Build history of the part. All positions in model axes, mm. A direction names the side the tool comes from. Coordinates: 2 decimals unless noted, no trailing zeros. Loops run counter-clockwise (first coordinate to the right, second up) from the corner with the lowest first, then second, coordinate; pieces in that order, holes last. Notation, with made-up numbers: (59, 86) - (94, 86) arc R18 ccw to (94, 113) - close; hole circle Ø1 at (3, -28.75). An arc over 180 degrees is marked (long way). One line per item, written item: value.
```python
from build123d import *

# Parameters (mm, degrees)
BOSS_EXTRUDE2_DEPTH = 45


with BuildPart() as part:
    # Sketch1 → Boss-Extrude2 (new body)
    with BuildSketch(Plane.XY):
        Polygon((-15.25, 11.25), (-14.75, 11.75), (-8, 11.75), (-8, 10.25), (-5, 10.25), (-5, 11.75), (5, 11.75), (5, 10.25), (8, 10.25), (8, 11.75), (14.75, 11.75), (15.25, 11.25), (15.25, 2.78649269), (13.75, 2.78649269), (13.75, -2.78649269), (15.25, -2.78649269), (15.25, -11.25), (14.75, -11.75), (8, -11.75), (8, -10.25), (5, -10.25), (5, -11.75), (-5, -11.75), (-5, -10.25), (-8, -10.25), (-8, -11.75), (-14.75, -11.75), (-15.25, -11.25), (-15.25, -2.78649269), (-13.75, -2.78649269), (-13.75, 2.78649269), (-15.25, 2.78649269), align=None)
    extrude(amount=BOSS_EXTRUDE2_DEPTH)


solid = part.part
```
Item 1: Pull direction Y, two halves, no side cores. Call faces 6 (the face through (15, 2.786, 22)), 7 (the face through (-13.75, 0, 22)), 8 (the face through (-11, 11.75, 22)), 9 (the face through (-5, -11, 22)): released by +Y, released by -Y, zero draft, split by the parting line, or undercut.
Check result:
face 6: undercut
face 7: undercut
face 8: released by +Y
face 9: zero draft
Item 2: Probe probe 1 along X at (y, z) = (-0.25, 36); probe 2 along Y at (x, z) = (-7, 4.5). List the from-to ranges inside material, lowest first. Write a range as from..to.
Check result:
probe 1: x = -13.75..13.75
probe 2: y = -10.25..10.25
Item 3: Cut at C-C, the plane x = -7. Write the cut outline in (y, z), then the cut area to 4 significant figures.
Check result:
outline: (-10.25, 0) - (10.25, 0) - (10.25, 45) - (-10.25, 45) - close
area: 922.5 mm^2
Item 4: Drop flat-ended pins along their axis: P1, Ø1.5, axis at x = -6.5, z = 27.5, coming from the -Y side; P2, Ø1.5, axis at x = 6.5, z = 26, coming from the +Y side; P3, Ø1.7, axis at y = 1, z = 25.5, coming from the +X side. Give the stop position or say it passes through.
Check result:
P1: stops at y = -10.25
P2: stops at y = 10.25
P3: stops at x = 13.75
Item 5: Cut at B-B, the plane y = 0. Write the cut outline in (x, z), then the cut area to 3 significant figures.
Check result:
outline: (-13.75, 0) - (13.75, 0) - (13.75, 45) - (-13.75, 45) - close
area: 1,240 mm^2
Item 6: Tool access for faces 1 (the face through (-6, -10.25, 22)), 2 (the face through (-5, 11, 22)), 3 (the face through (-15, -2.786, 22)), 4 (the face through (14, -2.786, 22)), 5 (the face through (11, -11.75, 22)): list every direction of +Z, -Z, +X, -X, +Y, -Y with a clear straight run to the whole face (end or side of a thin tool).
Check result:
face 1: +Z, -Z, -Y
face 2: +Z, -Z, +Y
face 3: +Z, -Z, -X
face 4: +Z, -Z, +X
face 5: +Z, -Z, +X, -X, -Y
